Here's the drawing with two shaded views (mm, measured from the low corner). I have some questions. A direction names the side the tool comes from. Give positions to 0.01 mm unless a question says otherwise; leave off trailing zeros. Answer in a Markdown table with one row per item. Add a question column.
Item 1: Which directions (+Z, -Z, +X, -X, +Y, -Y) give clear straight access to the entire face, cutting with the end or side of a thin tool? Please do the marked faces 4, 5, 6 and 7.
Item 2: If we section it at A-A (x = 2): Give the number of separate pieces and of enclosed holes in the cut face, then the cut area to 3 significant figures.
Item 3: We'd pull the mould along Z, two halves only. Please class the marked faces 1, 2 and 3: released by +Z, released by -Z, zero draft, split by the parting line, or undercut.
Item 4: If I drill on line 1 (Y direction, x = 11.75, z = 20) (1 decimal); line 2 (Z direction, x = 3.25, y = 22.5) (1 decimal); line 3 (Y direction, x = 10.25, z = 20) (1 decimal), over which ranges is the centre line in solid material (lowest first)?
Item 5: For P1, Ø3, axis at x = 13, z = 32, coming from the -Y side; P2, Ø1.5, axis at y = 15.5, z = 6.5, coming from the -X side; P3, Ø2, axis at x = 1.5, z = 29.5, coming from the +Y side, each with a flat end and sliding along its axis, tell me the tip position at first contact or that it passes through.
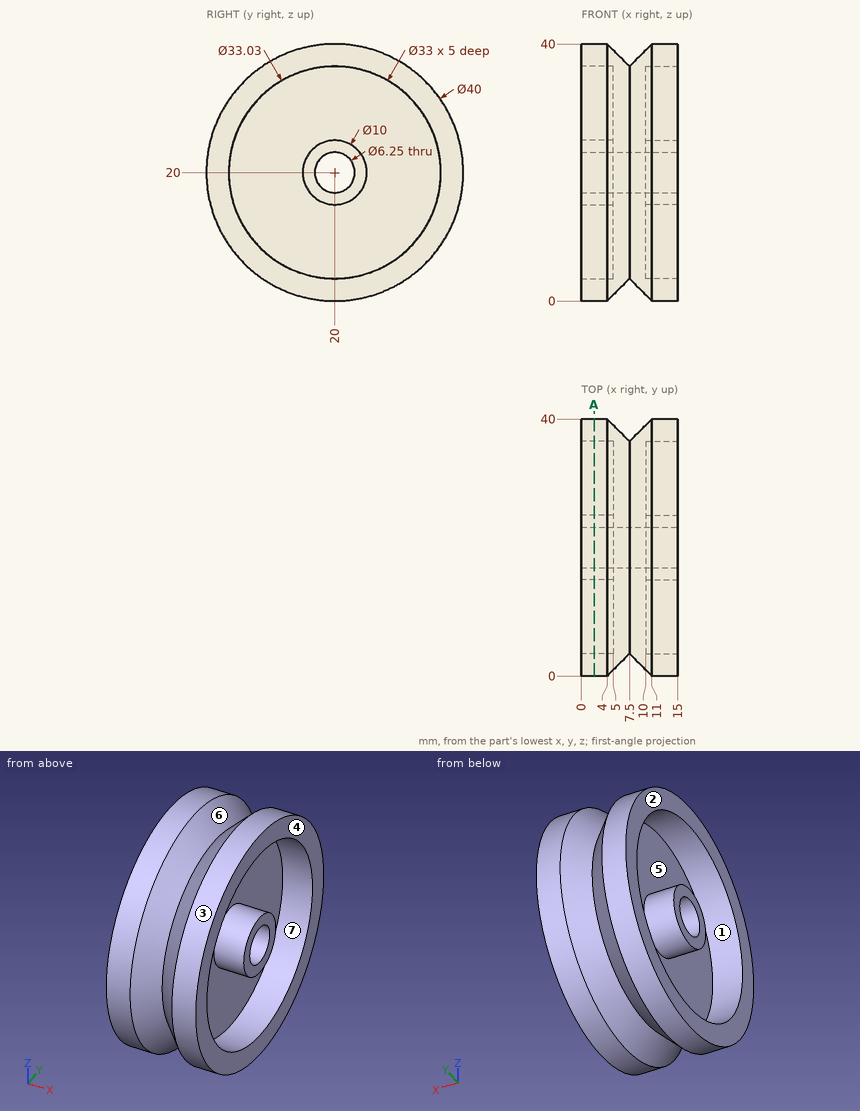
Recorded:
| question | item | result |
|---|---|---|
| 1 | face 4 | +Z, -Z, +X, +Y, -Y |
| 1 | face 5 | -X |
| 1 | face 6 | none |
| 1 | face 7 | +X |
| 2 | separate pieces | 2 |
| 2 | enclosed holes | 2 |
| 2 | area | 449 mm^2 |
| 3 | face 1 | undercut |
| 3 | face 2 | zero draft |
| 3 | face 3 | split by the parting line |
| 4 | line 1 | y = 0 to 3.5, 15 to 16.9, 23.1 to 25, 36.5 to 40 |
| 4 | line 2 | z = 0.2 to 3.7, 15.7 to 18.1, 21.9 to 24.3, 36.3 to 39.8 |
| 4 | line 3 | y = 0.7 to 3.5, 15 to 16.9, 23.1 to 25, 36.5 to 39.3 |
| 5 | P1 | stops at y = 2.98 |
| 5 | P2 | stops at x = 5 |
| 5 | P3 | stops at y = 38.1 |
